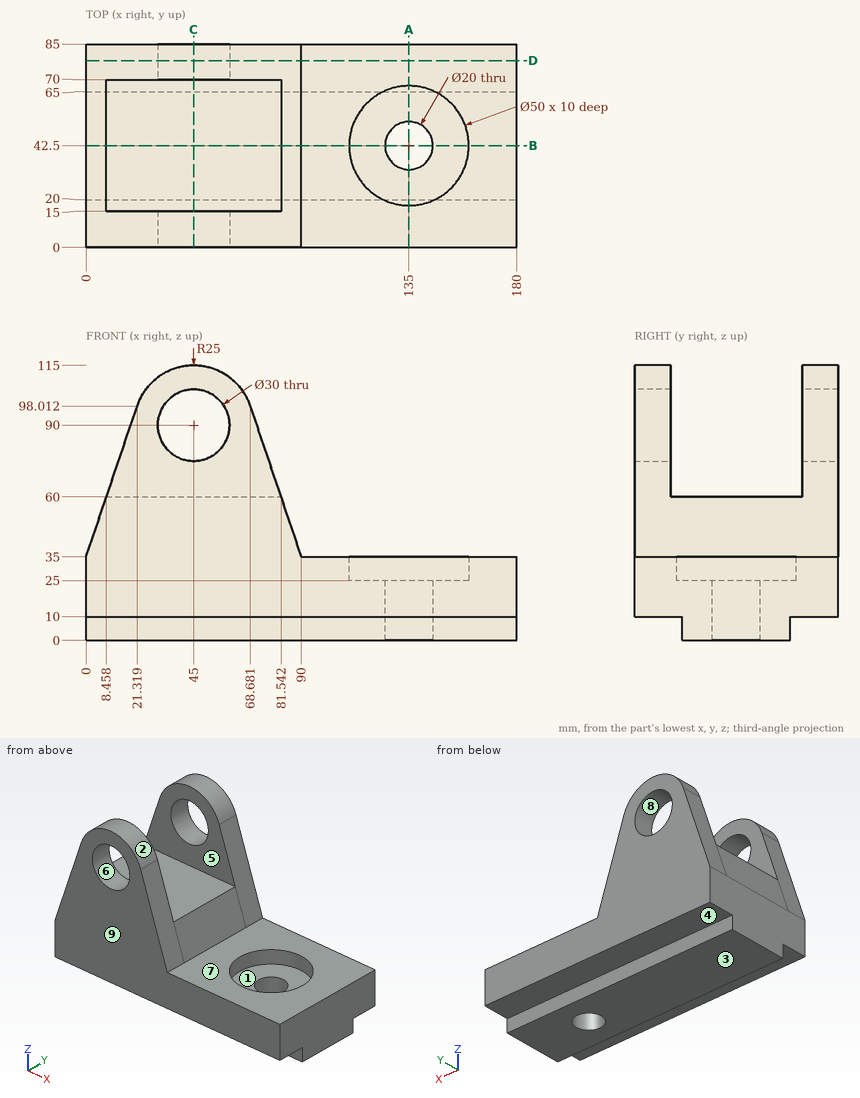
The figure shows three views and two pictorial views of one solid part (mm, origin at its lowest corner). Answer the questions. A direction names the side the tool comes from. Give positions to 0.01 mm unless a question says otherwise; leave off trailing zeros. Write each loop counter-clockwise with the first axis right and the second up, starting at its lowest first coordinate (ties: lowest second). Pieces come first, ordered by that corner, then holes. Notation, with made-up numbers: (74, 47) - (80, 47) arc R21 cw to (80, 80) - close; hole circle Ø11 at (80.5, 48). An arc over 180 degrees is marked (long way). Return JSON: item names as keys, results as strings.
Q1. Consider line 1 along Y through (x, z) = (135, 28); line 2 along Y through (x, z) = (135, 15); line 3 along Z through (x, y) = (45, 81.75). Determine where each line is inside the solid, lowest interval first. Write a range as [from, to].
Reply:
{"line 1": "[0, 17.5], [67.5, 85]", "line 2": "[0, 32.5], [52.5, 85]", "line 3": "[10, 75], [105, 115]"}
Q2. A cutting plane is placed at D-D, the plane y = 78. Determine the outline of the cut face in (x, z).
Reply:
{"outline": "(0, 10) - (180, 10) - (180, 35) - (90, 35) - (68.68, 98.01) arc R25 ccw to (21.32, 98.01) - (0, 35) - close; hole circle Ø30 at (45, 90)"}
Q3. A cutting plane is placed at B-B, the plane y = 42.5. Determine the outline of the cut face in (x, z), and give its area (3 significant figures).
Reply:
{"outline": "(0, 0) - (125, 0) - (125, 25) - (110, 25) - (110, 35) - (90, 35) - (81.54, 60) - (8.46, 60) - (0, 35) - close; (145, 0) - (180, 0) - (180, 35) - (160, 35) - (160, 25) - (145, 25) - close", "area": "7,340 mm²"}
Q4. For a pull along Z with two mould halves and no side action, classify the marked faces 6, 7, 8 and 9 as released by +Z, released by -Z, zero draft, split by the parting line, or undercut.
Reply:
{"face 6": "undercut", "face 7": "released by +Z", "face 8": "undercut", "face 9": "zero draft"}
Q5. Given P1, Ø1, axis at x = 101.5, y = 17, coming from the +Z side; P2, Ø4, axis at x = 56.5, y = 13, coming from the -Z side; P3, Ø10, axis at y = 67, z = 66, coming from the +X side (1 decimal); P4, Ø18, axis at x = 45, z = 90, coming from the +Y side, each flat-ended and moving along its own axis, determine where each tip first touches the part or whether it passes through.
Reply:
{"P1": "z = 35", "P2": "z = 10", "P3": "x = 80.9", "P4": "through"}
Q6. A cutting plane is placed at C-C, the plane x = 45. Determine the outline of the cut face in (y, z), and give its area (3 significant figures).
Reply:
{"outline": "(0, 10) - (20, 10) - (20, 0) - (65, 0) - (65, 10) - (85, 10) - (85, 75) - (70, 75) - (70, 60) - (15, 60) - (15, 75) - (0, 75) - close; (0, 105) - (15, 105) - (15, 115) - (0, 115) - close; (70, 105) - (85, 105) - (85, 115) - (70, 115) - close", "area": "5,450 mm²"}
Q7. A cutting plane is placed at A-A, the plane x = 135. Determine the outline of the cut face in (y, z).
Reply:
{"outline": "(0, 10) - (20, 10) - (20, 0) - (32.5, 0) - (32.5, 25) - (17.5, 25) - (17.5, 35) - (0, 35) - close; (52.5, 0) - (65, 0) - (65, 10) - (85, 10) - (85, 35) - (67.5, 35) - (67.5, 25) - (52.5, 25) - close"}
Q8. For the marked faces 1, 2, 3, 4 and 5, determine the directions among +Z, -Z, +X, -X, +Y, -Y from which every point of the face is accessible in a straight line to the end or side of a thin tool.
Reply:
{"face 1": "+Z", "face 2": "+Z, +Y, -Y", "face 3": "-Z, +X, -X, +Y, -Y", "face 4": "-Z, +X, -X, +Y", "face 5": "+Z, +X, -X"}
